Read the model definition and answer for the solid it produces. Units are mm, in the model's axes. Face numbers are marked on the shaded views. A direction names the side the tool comes from. Round coordinates to 2 decimals unless told otherwise and drop trailing zeros. Order: outer loops, then holes, each group sorted by start corner. A loop starts at its lowest first (then second) coordinate and runs counter-clockwise, first axis right, second up.
from build123d import *
from build123d.topology import SkipClean

# Parameters (mm, degrees)
BASE_DISC_SKETCH_75_R = 37.5
BASE_DISC_75X3_DEPTH  = 3
HUB_AND_BORE_SKETCH_R = 12.5
HUB_BOSS_DEPTH        = 16
SHAFT_BORE_DEPTH      = 23
HUB_FILLET_R6_R       = 6
VANES_6X_DEPTH        = 14
VANE_FILLETS_R2_R     = 2


with BuildPart() as part:
    # Base Disc Sketch _75 → Base Disc _75x3 (new body)
    with BuildSketch(Plane(origin=(0, 0, 0), x_dir=(1, 0, 0), z_dir=(0, 1, 0))):
        with Locations(Location((0, 0, 0), (0, 0, 270))):
            Circle(BASE_DISC_SKETCH_75_R)
    extrude(amount=BASE_DISC_75X3_DEPTH)

    # Hub and Bore Sketch → Hub Boss (add)
    with BuildSketch(Plane.XZ):
        with Locations(Location((0, 0, 0), (0, 0, 270))):
            Circle(HUB_AND_BORE_SKETCH_R)
    extrude(amount=HUB_BOSS_DEPTH)

    # Sketch2_3 → Shaft Bore (cut, symmetric)
    with BuildSketch(Plane.XZ):
        with BuildLine():
            Line((-2.5, 8.838348415), (2.5, 8.838348415))
            Line((2.5, 8.838348415), (2.5, 6.538348415))
            ThreePointArc((2.5, 6.538348415), (0, -7), (-2.5, 6.538348415))
            Line((-2.5, 6.538348415), (-2.5, 8.838348415))
        make_face()
    extrude(amount=SHAFT_BORE_DEPTH, both=True, mode=Mode.SUBTRACT)

    # Hub Fillet R6
    hub_fillet_r6_edges = [part.edges().sort_by_distance(p)[0] for p in [
        (0, 0, 12.5),
    ]]
    fillet(hub_fillet_r6_edges, radius=HUB_FILLET_R6_R)

    # Vane Profiles Sketch 6x → Vanes 6x (add)
    with SkipClean():  # the faces are left unmerged after this step: merging them gives an invalid solid
        with BuildSketch(Plane(origin=(0, 3, 0), x_dir=(1, 0, 0), z_dir=(0, 1, 0))):
            with BuildLine():
                Line((13.151074283, 8.81994991), (12.093810893, 13.81994991))
                ThreePointArc((12.093810893, 13.81994991), (26.507335187, 10.054378643), (37.5, 0))
                ThreePointArc((37.5, 0), (37.416199333, -2.505599224), (37.165171868, -5))
                ThreePointArc((37.165171868, -5), (26.987316196, 5.088454065), (13.151074283, 8.81994991))
            make_face()
            with BuildLine():
                Line((14.213837824, -6.979189461), (18.015333148, -3.563572506))
                ThreePointArc((18.015333148, -3.563572506), (21.961014917, -17.928836338), (18.75, -32.475952642))
                ThreePointArc((18.75, -32.475952642), (16.538187087, -33.656178747), (14.252458915, -34.685982974))
                ThreePointArc((14.252458915, -34.685982974), (17.900388584, -20.827474373), (14.213837824, -6.979189461))
            make_face()
            with BuildLine():
                Line((1.062763541, -15.799139371), (5.921522255, -17.383522417))
                ThreePointArc((5.921522255, -17.383522417), (-4.54632027, -27.98321498), (-18.75, -32.475952642))
                ThreePointArc((-18.75, -32.475952642), (-20.878012246, -31.150579524), (-22.912712953, -29.685982974))
                ThreePointArc((-22.912712953, -29.685982974), (-9.086927612, -25.915928438), (1.062763541, -15.799139371))
            make_face()
            with BuildLine():
                Line((-13.151074283, -8.81994991), (-12.093810893, -13.81994991))
                ThreePointArc((-12.093810893, -13.81994991), (-26.507335187, -10.054378643), (-37.5, 0))
                ThreePointArc((-37.5, 0), (-37.416199333, 2.505599224), (-37.165171868, 5))
                ThreePointArc((-37.165171868, 5), (-26.987316196, -5.088454065), (-13.151074283, -8.81994991))
            make_face()
            with BuildLine():
                Line((-14.213837824, 6.979189461), (-18.015333148, 3.563572506))
                ThreePointArc((-18.015333148, 3.563572506), (-21.961014917, 17.928836338), (-18.75, 32.475952642))
                ThreePointArc((-18.75, 32.475952642), (-16.538187087, 33.656178747), (-14.252458915, 34.685982974))
                ThreePointArc((-14.252458915, 34.685982974), (-17.900388584, 20.827474373), (-14.213837824, 6.979189461))
            make_face()
            with BuildLine():
                Line((-1.062763541, 15.799139371), (-5.921522255, 17.383522417))
                ThreePointArc((-5.921522255, 17.383522417), (4.54632027, 27.98321498), (18.75, 32.475952642))
                ThreePointArc((18.75, 32.475952642), (20.878012246, 31.150579524), (22.912712953, 29.685982974))
                ThreePointArc((22.912712953, 29.685982974), (9.086927612, 25.915928438), (-1.062763541, 15.799139371))
            make_face()
        extrude(amount=VANES_6X_DEPTH)

    # Vane Fillets R2
    vane_fillets_r2_edges = [part.edges().sort_by_distance(p)[0] for p in [
        (12.622442588, 3, -11.31994991),
        (16.114585486, 3, 5.271380984),
        (3.492142898, 3, 16.591330894),
        (-12.622442588, 3, 11.31994991),
        (-16.114585486, 3, -5.271380984),
        (-3.492142898, 3, -16.591330894),
    ]]
    fillet(vane_fillets_r2_edges, radius=VANE_FILLETS_R2_R)


solid = part.part
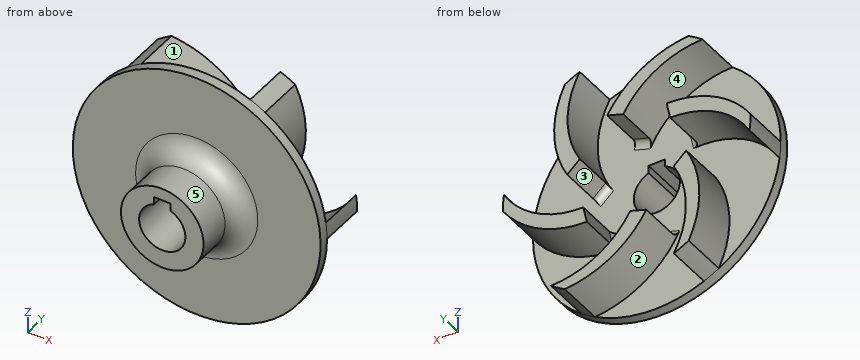
Q1. Straight lines are drawn through the part: probe 1 along X at (y, z) = (-11.75, 0); probe 2 along Y at (x, z) = (25.5, -2.5); probe 3 along Y at (x, z) = (17.5, 10.5). For each, find the intervals that lie inside material, in ascending order.
Outcome:
probe 1: x = -12.5 to -7, 7 to 12.5
probe 2: y = 0 to 3
probe 3: y = 0 to 17
Q2. A cutting plane is placed at C-C, the plane y = -3.5. Give the vertices of the cut face in (x, z), plus the area to 3 significant figures.
Outcome:
outline: circle Ø26.09 at (0, 0); hole (-2.5, 6.54) arc R7 ccw (long way) to (2.5, 6.54) - (2.5, 8.84) - (-2.5, 8.84) - close
area: 371 mm2
Q3. A cutting plane is placed at A-A, the plane y = -10. Give the vertices of the cut face in (x, z), plus the area to 3 significant figures.
Outcome:
outline: circle Ø25 at (0, 0); hole (-2.5, 6.54) arc R7 ccw (long way) to (2.5, 6.54) - (2.5, 8.84) - (-2.5, 8.84) - close
area: 327 mm2
Q4. A cutting plane is placed at B-B, the plane x = 0. Give the vertices of the cut face in (y, z), plus the area to 3 significant figures.
Outcome:
outline: (-16, -12.5) - (-6, -12.5) arc R6 cw to (0, -18.5) - (0, -37.5) - (3, -37.5) - (3, -24.59) - (17, -24.59) - (17, -17.48) - (3, -17.48) - (3, -7) - (-16, -7) - close; (-16, 8.84) - (3, 8.84) - (3, 17.48) - (17, 17.48) - (17, 24.59) - (3, 24.59) - (3, 37.5) - (0, 37.5) - (0, 18.5) arc R6 cw to (-6, 12.5) - (-16, 12.5) - close
area: 539 mm2
Q5. Flat-ended cylindrical pins translate along their axes: pin 1 (5 mm diameter, centred on y = -8.5, z = -17, fed in from +X); pin 2 (8 mm diameter, centred on y = 10.5, z = -28, fed in from -X); pin 3 (5 mm diameter, centred on y = -7, z = -12.5, fed in from +X); pin 4 (1.2 mm diameter, centred on y = -7, z = 7, fed in from +X). Find the tip coordinate at first contact, or state that the pin passes through.
Outcome:
pin 1: passes through
pin 2: stops at x = -21.52
pin 3: stops at x = 7.5
pin 4: stops at x = 10.74
Q6. For the marked faces 1, 2, 3, 4 and 5, determine the directions among +Z, -Z, +X, -X, +Y, -Y from which every point of the face is accessible in a straight line to the end or side of a thin tool.
Outcome:
face 1: +Z, +Y
face 2: -Z, +Y
face 3: +Y
face 4: -X, +Y
face 5: -Y
